```python
from build123d import *

# Parameters (mm, degrees)
SKETCH1_W                = 40
SKETCH1_H                = 30
BOSS_EXTRUDE1_DEPTH      = 3
M4_CLEARANCE_HOLE1_D     = 4.8
M4_CLEARANCE_HOLE1_DEPTH = 10.1
M4_CLEARANCE_HOLE1_TIP   = 1.442065486


with BuildPart() as part:
    # Sketch1 → Boss-Extrude1 (new body)
    with BuildSketch(Plane(origin=(0, 0, 0), x_dir=(1, 0, 0), z_dir=(0, 1, 0))):
        Rectangle(SKETCH1_W, SKETCH1_H)
    extrude(amount=BOSS_EXTRUDE1_DEPTH)

    # M4 Clearance Hole1
    with Locations(Plane(origin=(-8, 0, 0.030903026), x_dir=(0, 0, -1), z_dir=(0, -1, 0))):
        with Locations((0, 0), (0, 16)):
            Hole(M4_CLEARANCE_HOLE1_D / 2, depth=M4_CLEARANCE_HOLE1_DEPTH)
            with Locations((0, 0, -(M4_CLEARANCE_HOLE1_DEPTH + M4_CLEARANCE_HOLE1_TIP / 2))):  # 118° drill point
                Cone(0, M4_CLEARANCE_HOLE1_D / 2, M4_CLEARANCE_HOLE1_TIP, mode=Mode.SUBTRACT)


solid = part.part
```
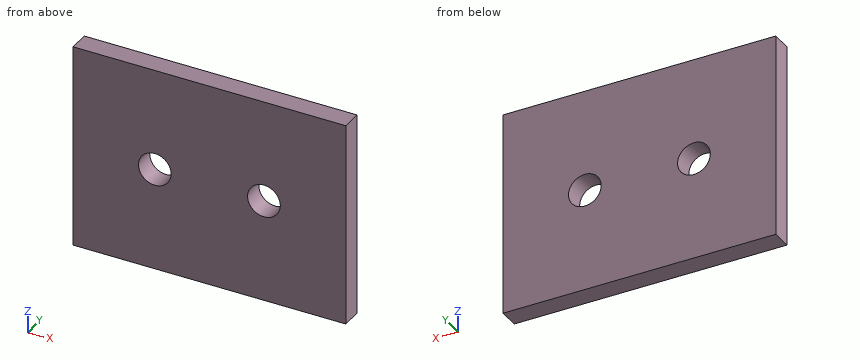
CAD build for the part. Positions are in the model's coordinates, mm. Give positions to 0.01 mm unless a question says otherwise; leave off trailing zeros. Write each loop counter-clockwise with the first axis right and the second up, starting at its lowest first coordinate (ties: lowest second). Pieces come first, ordered by that corner, then holes. Notation, with made-up numbers: M 20,12 L 66,12 A17 ccw 66,32 Z; hole C -5.75,-25.75 d6. An arc over 180 degrees is marked long. Return JSON: item names as keys, results as strings. Group by question number.
(1) Band-saw the part on B-B (y = 1.5). Give the cut face in (x, z), and give its area (3 significant figures).
(2) Flat gauge pin, fed straight in: pin 1 Ø4.5 at (x, z) = (8, 0.03) entering from +Y. Where does the tip first touch, or does it go through?
(3) Band-saw the part on A-A (x = 8). Give the cut face in (y, z), and give its area (3 significant figures).
(4) Band-saw the part on C-C (z = 1.25). Give the cut face in (x, y).
(5) Drill centre lines: L1, parallel to X at y = 0.15, z = -1.5; L2, parallel to X at y = 0.9, z = -0.75; L3, parallel to Z at x = -8.5, y = 2.75. Where is each one in solid material? Low to high. Write a range as [from, to].
Entries:
{
 "1": {"outline": "M -20,-15 L 20,-15 L 20,15 L -20,15 Z; hole C -8,0.03 d4.8; hole C 8,0.03 d4.8", "area": "1,160 mm^2"},
 "2": {"pin 1": "passes through"},
 "3": {"outline": "M 0,-15 L 3,-15 L 3,-2.37 L 0,-2.37 Z; M 0,2.43 L 3,2.43 L 3,15 L 0,15 Z", "area": "75.6 mm^2"},
 "4": {"outline": "M -20,0 L -10.07,0 L -10.07,3 L -20,3 Z; M -5.93,0 L 5.93,0 L 5.93,3 L -5.93,3 Z; M 10.07,0 L 20,0 L 20,3 L 10.07,3 Z"},
 "5": {"L1": "x = [-20, -9.85], [-6.15, 6.15], [9.85, 20]", "L2": "x = [-20, -10.27], [-5.73, 5.73], [10.27, 20]", "L3": "z = [-15, -2.32], [2.38, 15]"}
}
